The listing builds one solid part. Answer for the finished solid, in the listing's coordinates (mm). A direction names the side the tool comes from. Coordinates: 2 decimals unless noted, no trailing zeros. Write each loop counter-clockwise with the first axis right and the second up, starting at its lowest first coordinate (ties: lowest second). Pieces come first, ordered by that corner, then holes.
from build123d import *

# Parameters (mm, degrees)
CHAMFER_1_SIZE           = 2
CHAMFER_2_SIZE           = 2
SKETCH_8_R               = 30
SKETCH_8_R_2             = 20
EXTRUDE_1_DEPTH          = 76
SKETCH_9_W               = 12
SKETCH_9_H               = 4.221215972
CUT_EXTRUDE_1_DEPTH      = 104.807514179
SKETCH_11_W              = 2.5
SKETCH_11_H              = 26.7
PATTERN_CIRCULAR_2_COUNT = 4
SKETCH_14_R              = 5.5
CUT_EXTRUDE_2_DEPTH      = 8
PATTERN_CIRCULAR_3_COUNT = 4


with BuildPart() as part:
    # 草图1 → 旋转1 (revolve)
    with BuildSketch(Plane(origin=(0, 0, 0), x_dir=(0, 0, -1), z_dir=(1, 0, 0)), mode=Mode.PRIVATE) as revolve_1_sk:
        Polygon((0, 21), (0, 40), (-51, 40), (-51, 50), (-76, 50), (-76, 30), (-16, 30), (-16, 21), align=None)
    revolve(revolve_1_sk.sketch.rotate(Axis((0, 0, 0), (0, 0, -1)), 90), axis=Axis((0, 0, 0), (0, 0, -1)))

    # 倒角1
    chamfer_1_edges = [part.edges().sort_by_distance(p)[0] for p in [
        (-40, 0, 51),
    ]]
    chamfer(chamfer_1_edges, length=CHAMFER_1_SIZE)

    # 倒角2
    chamfer_2_edges = [part.edges().sort_by_distance(p)[0] for p in [
        (-40, 0, 0),
    ]]
    chamfer(chamfer_2_edges, length=CHAMFER_2_SIZE)

    # 草图8 → 凸台-拉伸1 (add, through all)
    with BuildSketch(Plane.XY.offset(76)):
        Circle(SKETCH_8_R)
        Circle(SKETCH_8_R_2, mode=Mode.SUBTRACT)
    extrude(amount=-EXTRUDE_1_DEPTH)

    # 草图9 → 切除-拉伸1 (cut, through all)
    with BuildSketch(Plane(origin=(0, 0, 0), x_dir=(-1, 0, 0), z_dir=(0, 0, -1))):
        with Locations((0, 21.189392014)):
            Rectangle(SKETCH_9_W, SKETCH_9_H)
    extrude(amount=-CUT_EXTRUDE_1_DEPTH, mode=Mode.SUBTRACT)

    # 草图11 → M6 螺纹孔1 (revolve, cut)
    with BuildSketch(Plane(origin=(0, 23.3, 25.5), x_dir=(0, 0, -1), z_dir=(1, 0, 0))):
        with Locations((1.25, 13.35)):
            Rectangle(SKETCH_11_W, SKETCH_11_H)
    hole_wizard_m6_1 = revolve(axis=Axis((0, 16.95, 25.5), (0, 1, 0)), mode=Mode.SUBTRACT)

    # 阵列(圆周)2: M6 螺纹孔1 ×4 about axis
    pattern_circular_2_axis = Axis((0, 0, 0), (0, 0, 1))
    for i in range(1, PATTERN_CIRCULAR_2_COUNT):
        add(hole_wizard_m6_1.rotate(pattern_circular_2_axis, i * 360 / PATTERN_CIRCULAR_2_COUNT), mode=Mode.SUBTRACT)

    # 草图14 → 切除-拉伸2 (cut)
    with BuildSketch(Plane.ZY.offset(40)):
        with Locations((25.5, 0)):
            Circle(SKETCH_14_R)
    cut_extrude_2 = extrude(amount=-CUT_EXTRUDE_2_DEPTH, mode=Mode.SUBTRACT)

    # 阵列(圆周)3: 切除-拉伸2 ×4 about axis
    pattern_circular_3_axis = Axis((0, 0, 0), (0, 0, 1))
    for i in range(1, PATTERN_CIRCULAR_3_COUNT):
        add(cut_extrude_2.rotate(pattern_circular_3_axis, i * 360 / PATTERN_CIRCULAR_3_COUNT), mode=Mode.SUBTRACT)


solid = part.part
1. Section D-D on z = 38 is taken. Give the vertices of the cut face in (x, y), then the cut area to 3 significant figures.
Results found:
outline: circle Ø80 at (0, 0); hole (-6, 19.08) arc R20 ccw (long way) to (6, 19.08) - (6, 23.3) - (-6, 23.3) - close
area: 3,730 mm2
2. Find the intervals of material crossed by L1, parallel to Z at x = 0, y = 28.5; L2, parallel to Z at x = 0, y = -37.75; L3, parallel to X at y = 0, z = 34, in increasing order.
Results found:
L1: z = 0 to 23, 28 to 76
L2: z = 0 to 20, 31 to 76
L3: x = -40 to -20, 20 to 40
3. For a pull along Z with two mould halves and no side action, classify faces 1 (the flat face through (0, -23.3, 25)), 2 (the flat face through (16, -16, 0)), 3 (the cylindrical face through (47.69, -15.02, 63.68)) as pulls with the +Z half, pulls with the -Z half, needs draft (parallel to the pull), parting line crosses it, or undercut.
Results found:
face 1: undercut
face 2: pulls with the -Z half
face 3: needs draft
4. Section C-C on z = 67 is taken. Give the vertices of the cut face in (x, y), then the cut area to 3 significant figures.
Results found:
outline: circle Ø100 at (0, 0); hole (-6, 19.08) arc R20 ccw (long way) to (6, 19.08) - (6, 23.3) - (-6, 23.3) - close
area: 6,550 mm2
5. Flat-ended cylindrical pins translate along their axes: P1, Ø12, axis at y = 19, z = 52.5, coming from the -X side; P2, Ø3.5, axis at x = 2.5, z = 24.5, coming from the -Y side; P3, Ø10, axis at x = -39.5, y = -37.5, coming from the -Z side. Find the tip coordinate at first contact, or state that the pin passes through.
Results found:
P1: stops at x = -48.28
P2: stops at y = -32
P3: stops at z = 51
6. A tool of negligible diameter and unlimited length cuts with its end or side. For faces 4 (the flat face through (32, 1, 28)), 5 (the flat face through (1, -32, 28)), 6 (the cylindrical face through (-28, 0, 28)), 7 (the flat face through (11, -41, 51)), 8 (the flat face through (0, 23.3, 37)), from which of +Z, -Z, +X, -X, +Y, -Y can it reach the whole face along a straight path? Write none if from no direction.
Results found:
face 4: +X
face 5: -Y
face 6: -X
face 7: -Z
face 8: +Z, -Z
7. Section A-A on x = 0 is taken. State how many separate pieces and enclosed holes the cut face has, then the cut area to 3 significant figures.
Results found:
separate pieces: 3
enclosed holes: 0
area: 3,030 mm2
